Here's the drawing with two shaded views (mm, measured from the low corner). I have some questions. A direction names the side the tool comes from. Give positions to 0.01 mm unless a question says otherwise; leave off trailing zeros. Loops run counter-clockwise (first coordinate to the right, second up) from the corner with the lowest first, then second, coordinate; pieces in that order, holes last. Notation, with made-up numbers: M -3.5,-35.75 L 50.5,-35.75 A14 ccw 50.5,-24.75 Z; hole C -2.75,32.25 d6. An arc over 180 degrees is marked long. Answer in a Markdown table with one row per item. Add a question column.
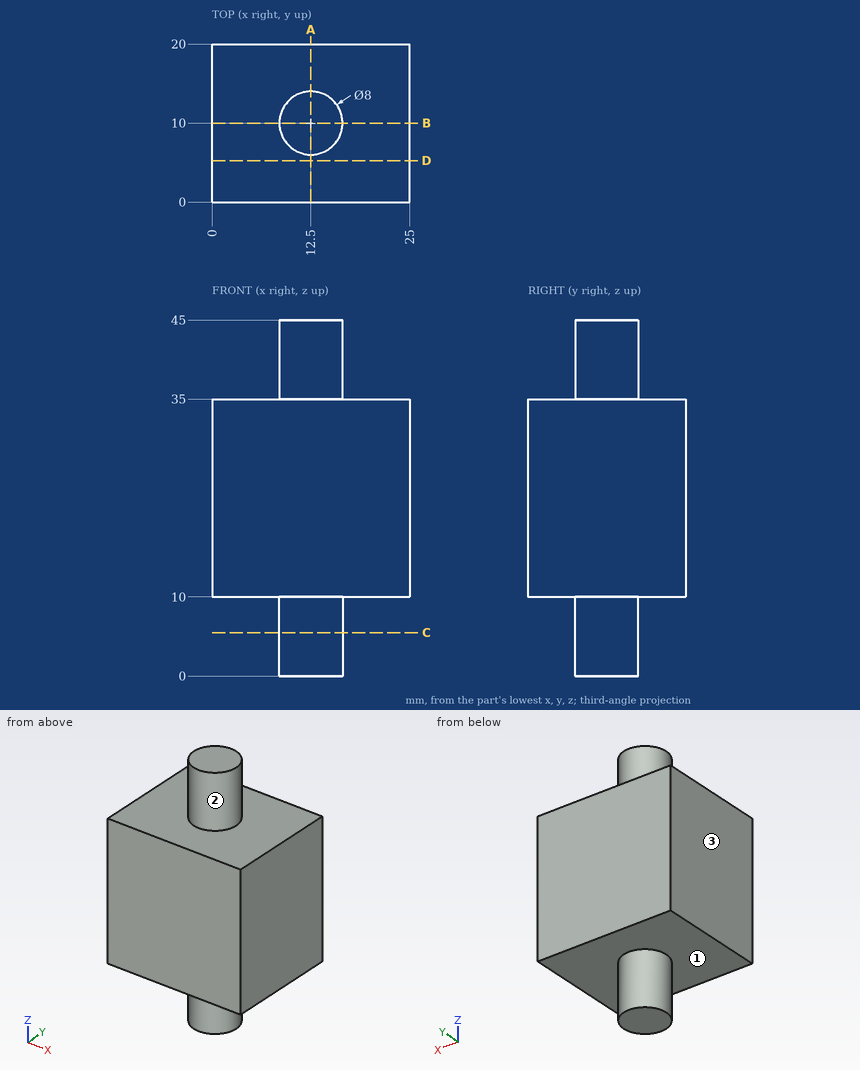
Item 1: Suppose I cut it at C-C (z = 5.5). List the corners of the cut face in (x, y) for me, then the cut area to 3 significant figures.
Item 2: Suppose I cut it at D-D (y = 5.25). List the corners of the cut face in (x, z) for me.
Item 3: I need wall thicknesses on L1, parallel to Z at x = 6.5, y = 16.75; L2, parallel to Y at x = 14, z = 8; L3, parallel to X at y = 7, z = 36.5. Which ranges of each line are inside material? Lowest first, please.
Item 4: Suppose I cut it at A-A (x = 12.5). List the corners of the cut face in (y, z) for me.
Item 5: Suppose I cut it at B-B (y = 10). List the corners of the cut face in (x, z) for me.
Item 6: For P1, Ø6, axis at x = 15.5, y = 7.5, coming from the -Z side; P2, Ø1.5, axis at x = 9.5, y = 15.5, coming from the -Z side; P3, Ø3, axis at x = 18, y = 13.5, coming from the +Z side, each with a flat end and sliding along its axis, tell me the tip position at first contact or that it passes through.
Item 7: For the marked faces 1, 2 and 3, which set-ups out of +Z, -Z, +X, -X, +Y, -Y let a thin tool reach every point of the face, with its end or its side?
Values found:
| question | item | result |
|---|---|---|
| 1 | outline | C 12.5,10 d8 |
| 1 | area | 50.3 mm² |
| 2 | outline | M 0,10 L 25,10 L 25,35 L 0,35 Z |
| 3 | L1 | 10 to 35 |
| 3 | L2 | 6.29 to 13.71 |
| 3 | L3 | 9.85 to 15.15 |
| 4 | outline | M 0,10 L 6,10 L 6,0 L 14,0 L 14,10 L 20,10 L 20,35 L 14,35 L 14,45 L 6,45 L 6,35 L 0,35 Z |
| 5 | outline | M 0,10 L 8.5,10 L 8.5,0 L 16.5,0 L 16.5,10 L 25,10 L 25,35 L 16.5,35 L 16.5,45 L 8.5,45 L 8.5,35 L 0,35 Z |
| 6 | P1 | z = 0 |
| 6 | P2 | z = 10 |
| 6 | P3 | z = 35 |
| 7 | face 1 | -Z |
| 7 | face 2 | +Z |
| 7 | face 3 | +Z, -Z, -X, +Y, -Y |
